Geometry: final body of the model. Coordinates: model frame, mm. Face numbers are marked on the shaded views. A direction names the side the tool comes from. Round coordinates to 2 decimals unless told otherwise and drop trailing zeros. Order: outer loops, then holes, each group sorted by start corner. A loop starts at its lowest first (then second) coordinate and runs counter-clockwise, first axis right, second up. Notation, with made-up numbers: M -11,53 L 20,53 A24 ccw 20,84 Z; hole C -14.75,-23 d3. An arc over 180 degrees is marked long. Return JSON: item names as keys, results as strings. Group by question number.
Q1. Access query for the marked faces 1, 2, 3, 4 and 5. Directions: +Z, -Z, +X, -X, +Y, -Y. A direction counts if a zero-diameter tool reaches every point of the face in a straight line with its end or side. Return the directions, or none.
Q2. Cut plane A-A on x = -2. Output: boundary loops of the cut face in (y, z).
Q3. Ray query, probe 1 along Z at (x, y) = (1.5, 8); probe 2 along X at (y, z) = (23.5, 8); probe 3 along Z at (x, y) = (0.5, 47). Return the intervals inside material, ascending.
Q4. Contact query for flat-ended pins moving along their axis: pin 1 (8 mm diameter, centred on y = 9, z = 6, fed in from -X); pin 2 (5 mm diameter, centred on x = 0.5, z = -1.5, fed in from -Y); pin 3 (1 mm diameter, centred on x = -1.5, y = 38, fed in from -Z). Output: stop coordinate, or through.
Q5. Cut plane B-B on z = 19.5. Output: boundary loops of the cut face in (x, y).
Q6. Cut plane C-C on y = 9. Output: boundary loops of the cut face in (x, z), and give its area (3 significant figures).
```python
from build123d import *

# Parameters (mm, degrees)
SKETCH1_W           = 6.28
SKETCH1_H           = 55.78
BOSS_EXTRUDE1_DEPTH = 45
CUT_EXTRUDE1_DEPTH  = 72.737493684
SKETCH3_W           = 9.5
SKETCH3_H           = 59
BOSS_EXTRUDE2_DEPTH = 2.5
SKETCH4_W           = 11.5
SKETCH4_H           = 61
BOSS_EXTRUDE3_DEPTH = 2.5


with BuildPart() as part:
    # Sketch1 → Boss-Extrude1 (new body)
    with BuildSketch(Plane(origin=(0, 0, 0), x_dir=(1, 0, 0), z_dir=(0, 1, 0))):
        Rectangle(SKETCH1_W, SKETCH1_H)
    extrude(amount=BOSS_EXTRUDE1_DEPTH)

    # Sketch2 → Cut-Extrude1 (cut, through all)
    with BuildSketch(Plane.XY.offset(27.89)):
        Polygon((-3.14, 0), (3.14, 0), (3.14, 1.107333439), align=None)
    extrude(amount=-CUT_EXTRUDE1_DEPTH, mode=Mode.SUBTRACT)

    # Sketch3 → Boss-Extrude2 (add)
    with BuildSketch(Plane(origin=(0, 45, 0), x_dir=(1, 0, 0), z_dir=(0, 1, 0))):
        Rectangle(SKETCH3_W, SKETCH3_H)
    extrude(amount=BOSS_EXTRUDE2_DEPTH)

    # Sketch4 → Boss-Extrude3 (add)
    with BuildSketch(Plane(origin=(0, 47.5, 0), x_dir=(1, 0, 0), z_dir=(0, 1, 0))):
        Rectangle(SKETCH4_W, SKETCH4_H)
    extrude(amount=BOSS_EXTRUDE3_DEPTH)


solid = part.part
```
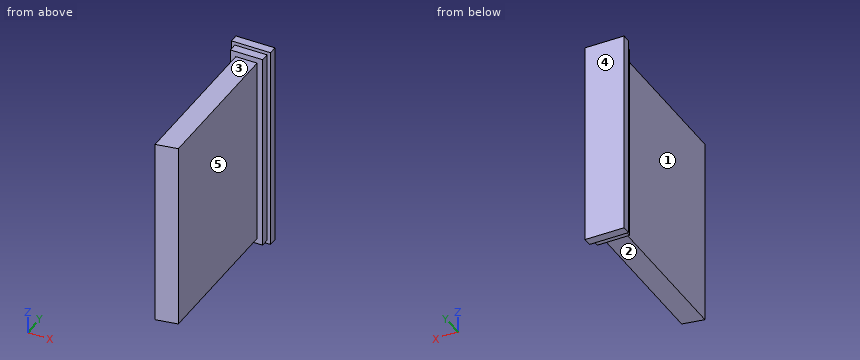
Result sheet:
{
 "1": {"face 1": "+Z, -Z, -X, -Y", "face 2": "-Z, +X, -X, -Y", "face 3": "+Z, +X, -X, -Y", "face 4": "+Z, -Z, +X, -X, +Y", "face 5": "+Z, -Z, +X, -Y"},
 "2": {"outline": "M 0.2,-27.89 L 45,-27.89 L 45,-29.5 L 47.5,-29.5 L 47.5,-30.5 L 50,-30.5 L 50,30.5 L 47.5,30.5 L 47.5,29.5 L 45,29.5 L 45,27.89 L 0.2,27.89 Z"},
 "3": {"probe 1": "z = -27.89 to 27.89", "probe 2": "x = -3.14 to 3.14", "probe 3": "z = -29.5 to 29.5"},
 "4": {"pin 1": "stops at x = -3.14", "pin 2": "stops at y = 0.2", "pin 3": "stops at z = -27.89"},
 "5": {"outline": "M -5.75,47.5 L -4.75,47.5 L -4.75,45 L -3.14,45 L -3.14,0 L 3.14,1.11 L 3.14,45 L 4.75,45 L 4.75,47.5 L 5.75,47.5 L 5.75,50 L -5.75,50 Z"},
 "6": {"outline": "M -3.14,-27.89 L 3.14,-27.89 L 3.14,27.89 L -3.14,27.89 Z", "area": "350 mm²"}
}
